```python
from build123d import *

# Parameters (mm, degrees)
SIDE_NOTCH_SKETCH_W  = 8.527366903
SIDE_NOTCH_SKETCH_H  = 6
SIDE_NOTCH_6X6_DEPTH = 9.5


with BuildPart() as part:
    # Pin Profile Sketch → Pin Body (revolve)
    with BuildSketch(Plane.XY, mode=Mode.PRIVATE) as pin_body_sk:
        Polygon((0, 0), (-2.5, 0), (-2.5, -5), (-6, -5), (-6, -10), (-3, -10), (-3, -35), (0, -35), align=None)
    revolve(pin_body_sk.sketch.rotate(Axis((0, -35, 0), (0, 1, 0)), 270), axis=Axis((0, -35, 0), (0, 1, 0)))

    # Side Notch Sketch → Side Notch 6x6 (cut, symmetric)
    with BuildSketch(Plane.XY):
        with Locations((4.263683452, -26)):
            Rectangle(SIDE_NOTCH_SKETCH_W, SIDE_NOTCH_SKETCH_H)
    extrude(amount=SIDE_NOTCH_6X6_DEPTH, both=True, mode=Mode.SUBTRACT)


solid = part.part
```
Geometry: final body of the model. Coordinates: model frame, mm. A direction names the side the tool comes from. Give positions to 0.01 mm unless a question says otherwise; leave off trailing zeros. Order: outer loops, then holes, each group sorted by start corner. A loop starts at its lowest first (then second) coordinate and runs counter-clockwise, first axis right, second up. Notation, with made-up numbers: (-10, -2.75) -> (29, -2.75) arc R14 ccw to (29, 12.25) -> close; hole circle Ø9 at (70.5, 65.5). An arc over 180 degrees is marked (long way). Write each question's results on one line, items separated by ' | '. Start each with the question number.
1) Draft query along Y for faces 4 (the flat face through (1, -10, 3)), 5 (the flat face through (1, -23, 0)), 6 (the cylindrical face through (-3, -23, 0)). Return one class per face: pulls with the +Y half, pulls with the -Y half, needs draft (parallel to the pull), parting line crosses it, or undercut.
2) Section B-B (y = -3). Return loops of the section in (x, z), then the cut area to 3 significant figures.
3) Section D-D (x = 5.25). Return loops of the section in (y, z).
4) Section C-C (z = -1.5). Return loops of the section in (x, y), then the cut area to 3 significant figures.
5) Set-up query: faces 1 (the cylindrical face through (-1.802, -7.535, -5.723)), 2 (the flat face through (0, -26, 0)), 3 (the cylindrical face through (2.44, -2.54, 0.54)). Return all of +Z, -Z, +X, -X, +Y, -Y with unobstructed straight access to the full face (end or side cutting, diameter ignored); none if empty.
6) Section A-A (z = 0). Return loops of the section in (x, y).
7) Line query: line 1 (Y direction, x = -4.5, z = 3); line 2 (Y direction, x = 1.5, z = 1.5); line 3 (Z direction, x = -2.75, y = -12.5). Output: solid intervals per line, ascending. Write a range as from..to.
8) First-contact query: pin 1 (5 mm diameter, centred on x = 3.5, y = -18.5, fed in from +Z); pin 2 (6.5 mm diameter, centred on y = -26, z = 0.5, fed in from +X); pin 3 (5 mm diameter, centred on x = -3.5, z = 5, fed in from -Y). Flat tips, straight axial feed; report the tip coordinate or a pass-through.
Calculated:
1) face 4: pulls with the -Y half | face 5: undercut | face 6: needs draft
2) outline: circle Ø5 at (0, 0) | area: 19.6 mm2
3) outline: (-10, -2.9) -> (-5, -2.9) -> (-5, 2.9) -> (-10, 2.9) -> close
4) outline: (-5.81, -10) -> (-2.6, -10) -> (-2.6, -35) -> (2.6, -35) -> (2.6, -29) -> (0, -29) -> (0, -23) -> (2.6, -23) -> (2.6, -10) -> (5.81, -10) -> (5.81, -5) -> (2, -5) -> (2, 0) -> (-2, 0) -> (-2, -5) -> (-5.81, -5) -> close | area: 192 mm2
5) face 1: +Y, -Y | face 2: +Z, -Z, +X | face 3: +Y
6) outline: (-6, -10) -> (-3, -10) -> (-3, -35) -> (3, -35) -> (3, -29) -> (0, -29) -> (0, -23) -> (3, -23) -> (3, -10) -> (6, -10) -> (6, -5) -> (2.5, -5) -> (2.5, 0) -> (-2.5, 0) -> (-2.5, -5) -> (-6, -5) -> close
7) line 1: -10..-5 | line 2: -35..-29, -23..0 | line 3: -1.2..1.2
8) pin 1: z = 2.83 | pin 2: x = 3 | pin 3: y = -10
